from build123d import *

# Parameters (mm, degrees)
SKETCH1_R           = 150
SKETCH1_R_2         = 80
BOSS_EXTRUDE1_DEPTH = 30
SKETCH2_R           = 9
CUT_EXTRUDE1_DEPTH  = 30
SKETCH3_R           = 9
CUT_EXTRUDE2_DEPTH  = 215.242852856
SKETCH4_R           = 13
CUT_EXTRUDE3_DEPTH  = 20


with BuildPart() as part:
    # Sketch1 → Boss-Extrude1 (new body)
    with BuildSketch(Plane.XY):
        Circle(SKETCH1_R)
        Circle(SKETCH1_R_2, mode=Mode.SUBTRACT)
    extrude(amount=BOSS_EXTRUDE1_DEPTH)

    # Sketch2 → Cut-Extrude1 (cut)
    with BuildSketch(Plane.XY.offset(30)):
        with Locations((0, 135)):
            Circle(SKETCH2_R)
        with Locations((116.913429511, 67.5)):
            Circle(SKETCH2_R)
        with Locations((116.913429511, -67.5)):
            Circle(SKETCH2_R)
        with Locations((0, -135)):
            Circle(SKETCH2_R)
        with Locations((-116.913429511, -67.5)):
            Circle(SKETCH2_R)
        with Locations((-116.913429511, 67.5)):
            Circle(SKETCH2_R)
    extrude(amount=-CUT_EXTRUDE1_DEPTH, mode=Mode.SUBTRACT)

    # Sketch3 → Cut-Extrude2 (cut, through all)
    with BuildSketch(Plane.XY.offset(30)):
        with Locations((0, 97.5)):
            Circle(SKETCH3_R)
        with Locations((84.437476869, 48.75)):
            Circle(SKETCH3_R)
        with Locations((84.437476869, -48.75)):
            Circle(SKETCH3_R)
        with Locations((0, -97.5)):
            Circle(SKETCH3_R)
        with Locations((-84.437476869, -48.75)):
            Circle(SKETCH3_R)
        with Locations((-84.437476869, 48.75)):
            Circle(SKETCH3_R)
    extrude(amount=-CUT_EXTRUDE2_DEPTH, mode=Mode.SUBTRACT)

    # Sketch4 → Cut-Extrude3 (cut)
    with BuildSketch(Plane.XY.offset(30)):
        with Locations((0, 97.5)):
            Circle(SKETCH4_R)
        with Locations((84.437476869, 48.75)):
            Circle(SKETCH4_R)
        with Locations((84.437476869, -48.75)):
            Circle(SKETCH4_R)
        with Locations((0, -97.5)):
            Circle(SKETCH4_R)
        with Locations((-84.437476869, -48.75)):
            Circle(SKETCH4_R)
        with Locations((-84.437476869, 48.75)):
            Circle(SKETCH4_R)
    extrude(amount=-CUT_EXTRUDE3_DEPTH, mode=Mode.SUBTRACT)


solid = part.part
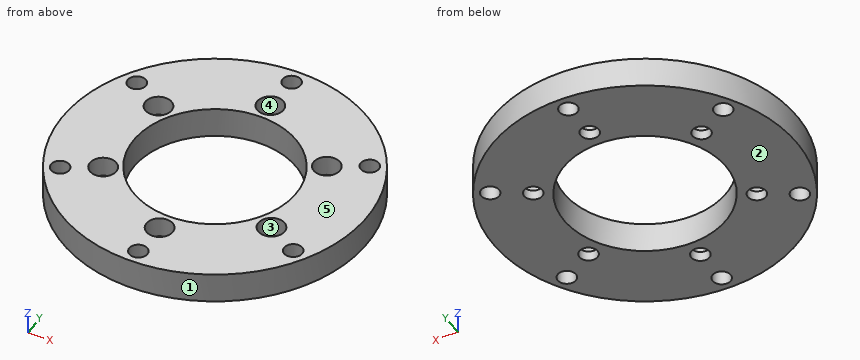
Design review of the part built by this model. Coordinates are the model's own, in mm. Face numbers are marked on the shaded views. A direction names the side the tool comes from. Coordinates: 2 decimals unless noted, no trailing zeros. Write each loop counter-clockwise with the first axis right and the second up, starting at its lowest first coordinate (ties: lowest second). Pieces come first, ordered by that corner, then holes. Notation, with made-up numbers: (40.25, 80.25) - (50.25, 80.25) arc R13 ccw to (50.25, 88.25) - close; hole circle Ø4 at (13.25, 32). An arc over 180 degrees is marked (long way). One line per item, written item: value.
1) To check wall thickness, follow probe 1 along Y at (x, z) = (-6, 24.5); probe 2 along X at (y, z) = (-46.5, 1.5); probe 3 along Y at (x, z) = (-83, 13.75). State the ranges of each line that lie inside material, in increasing order.
Answer sheet:
probe 1: y = -149.88 to -141.71, -128.29 to -109.03, -85.97 to -79.77, 79.77 to 85.97, 109.03 to 128.29, 141.71 to 149.88
probe 2: x = -142.61 to -93.15, -75.72 to -65.1, 65.1 to 75.72, 93.15 to 142.61
probe 3: y = -124.94 to -61.67, -35.83 to 35.83, 61.67 to 124.94
2) Add section C-C (y = 97.5). State the section outline as (x, z) points.
Answer sheet:
outline: (-113.99, 0) - (-9, 0) - (-9, 10) - (-13, 10) - (-13, 30) - (-113.99, 30) - close; (9, 0) - (113.99, 0) - (113.99, 30) - (13, 30) - (13, 10) - (9, 10) - close
3) For the marked faces 4 and 5, list the 3-axis set-ups (+Z, -Z, +X, -X, +Y, -Y) from which the entire face can be reached by the end or side of a thin tool; tool diameter is ignored.
Answer sheet:
face 4: +Z
face 5: +Z, +X, -X, +Y, -Y
4) Add section D-D (x = -48.5). State the section outline as (y, z) points, plus the area to 3 significant figures.
Answer sheet:
outline: (-141.94, 0) - (-63.62, 0) - (-63.62, 30) - (-141.94, 30) - close; (63.62, 0) - (141.94, 0) - (141.94, 30) - (63.62, 30) - close
area: 4,700 mm2
5) Insertion check: pin 1 (3 mm diameter, centred on y = 25, z = 23, fed in from +X); pin 2 (1 mm diameter, centred on x = 41.5, z = 4.5, fed in from +Y); pin 3 (10 mm diameter, centred on x = -92, z = 14.5, fed in from -Y); pin 4 (15.5 mm diameter, centred on x = -84.44, y = -48.75, fed in from +Z). Each pin has a flat end and moves straight along its axis. Give the tip position at first contact, or say it passes through.
Answer sheet:
pin 1: stops at x = 148.15
pin 2: stops at y = 144.29
pin 3: stops at y = -122.19
pin 4: passes through
6) Add section A-A (z = 23). Give the number of separate pieces and of enclosed holes in the cut face, plus the area to 3 significant figures.
Answer sheet:
separate pieces: 1
enclosed holes: 13
area: 45,900 mm2
7) Add section B-B (y = -48.75). State the section outline as (x, z) points.
Answer sheet:
outline: (-141.86, 0) - (-93.44, 0) - (-93.44, 10) - (-97.44, 10) - (-97.44, 30) - (-141.86, 30) - close; (-75.44, 0) - (-63.43, 0) - (-63.43, 30) - (-71.44, 30) - (-71.44, 10) - (-75.44, 10) - close; (63.43, 0) - (75.44, 0) - (75.44, 10) - (71.44, 10) - (71.44, 30) - (63.43, 30) - close; (93.44, 0) - (141.86, 0) - (141.86, 30) - (97.44, 30) - (97.44, 10) - (93.44, 10) - close
8) Mouldability with a two-part tool opening along Y and no side actions: class the marked faces 1, 2 and 3 as +Y half, -Y half, draft (parallel to the pull), parting line (faces both ways), or undercut.
Answer sheet:
face 1: parting line
face 2: draft
face 3: undercut
